Geometry: see drawing. Coordinates: mm, zero at the bounding-box minimum. A direction names the side the tool comes from. Coordinates: 2 decimals unless noted, no trailing zeros. Loops run counter-clockwise (first coordinate to the right, second up) from the corner with the lowest first, then second, coordinate; pieces in that order, holes last.
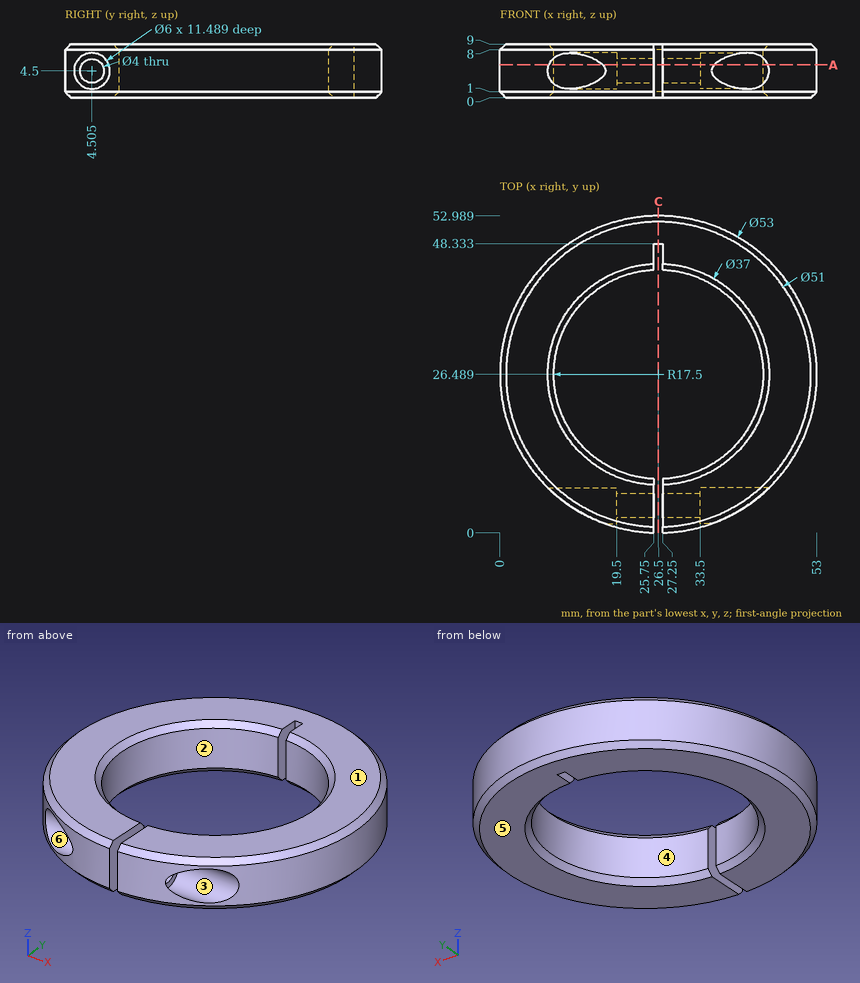
Item 1: Mould query, pull axis Z, two halves, no side actions, for the marked faces 1, 2 and 3. Classes: +Z half, -Z half, draft (parallel to the pull), parting line (faces both ways), or undercut.
Result:
face 1: +Z half
face 2: draft
face 3: undercut
Item 2: Section query C-C (x = 26.5). Output: boundary loops of the cut face in (y, z).
Result:
outline: (48.33, 0) - (51.99, 0) - (52.99, 1) - (52.99, 8) - (51.99, 9) - (48.33, 9) - close
Item 3: Contact query for flat-ended pins moving along their axis: P1, Ø3, axis at y = 24.5, z = 2.5, coming from the +X side (1 decimal); P2, Ø4, axis at x = 21.5, z = 3, coming from the +Y side; P3, Ø3, axis at x = 38, z = 4, coming from the -Y side; P4, Ø4, axis at x = 24.5, y = 40.5, coming from the +Z side. Output: stop coordinate, or through.
Result:
P1: stops at x = 53
P2: stops at y = 52.82
P3: stops at y = 6.74
P4: passes through
Item 4: Line query: L1, parallel to X at y = 26.5, z = 5.75; L2, parallel to Y at x = 24.5, z = 4.5 (1 decimal); L3, parallel to Y at x = 27, z = 5.25 (1 decimal). Output: solid intervals per line, ascending.
Result:
L1: x = 0 to 9, 44 to 53
L2: y = 0.1 to 2.5, 6.5 to 9.1, 43.9 to 52.9
L3: y = 48.3 to 53
Item 5: Section query A-A (z = 5.5). Count the separate pieces of the cut face and the enclosed holes in it, then the cut area to 3 significant figures.
Result:
separate pieces: 3
enclosed holes: 0
area: 1,100 mm2
Item 6: Reachability of the marked faces 4, 5 and 6 from +Z, -Z, +X, -X, +Y, -Y: full face, straight path, thin tool, end or side. Return the list, or none.
Result:
face 4: +Z, -Z
face 5: -Z, +X, -X, +Y, -Y
face 6: -X
